Verification items for this drawing (mm, ordinates from the low corner). A direction names the side the tool comes from. Coordinates: 2 decimals unless noted, no trailing zeros. Write each loop counter-clockwise with the first axis right and the second up, starting at its lowest first coordinate (ties: lowest second). Pieces come first, ordered by that corner, then holes. Notation, with made-up numbers: M -14,59 L 34,59 A19 ccw 34,93 Z; hole C -0.75,67.5 d7. An arc over 180 degrees is marked long. Write each question's results on one line, items separated by ' | '.
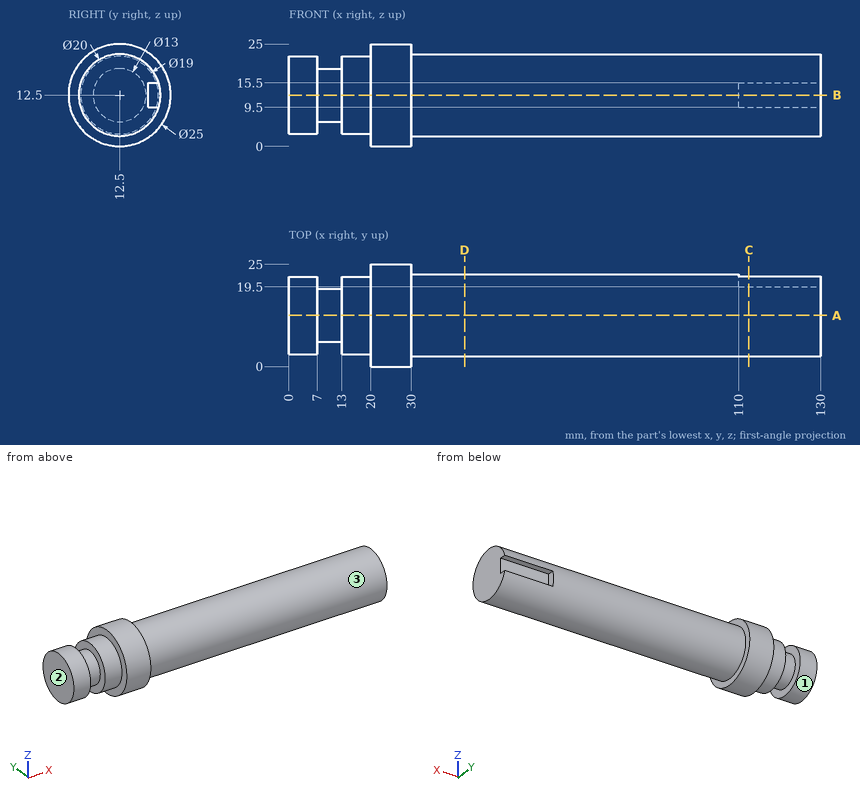
Q1. Sectioned sample at B-B on z = 12.5. Record the cut outline in (x, y).
Geometry check:
outline: M 0,3 L 7,3 L 7,6 L 13,6 L 13,3 L 20,3 L 20,0 L 30,0 L 30,2.5 L 130,2.5 L 130,19.5 L 110,19.5 L 110,22.5 L 30,22.5 L 30,25 L 20,25 L 20,22 L 13,22 L 13,19 L 7,19 L 7,22 L 0,22 Z
Q2. Sectioned sample at C-C on x = 112.5. Record the cut outline in (y, z), and give its area (3 significant figures).
Geometry check:
outline: M 19.5,9.5 L 19.5,15.5 L 22.04,15.5 A10 ccw long 22.04,9.5 Z | area: 297 mm2
Q3. Access from +Z, -Z, +X, -X, +Y, -Y to the whole of each face (thin tool, end or side, straight path). Record for the marked faces 1, 2 and 3.
Geometry check:
face 1: -X | face 2: +Z, -Z, -X, +Y, -Y | face 3: +X
Q4. Sectioned sample at A-A on y = 12.5. Record the cut outline in (x, z).
Geometry check:
outline: M 0,3 L 7,3 L 7,6 L 13,6 L 13,3 L 20,3 L 20,0 L 30,0 L 30,2.5 L 130,2.5 L 130,22.5 L 30,22.5 L 30,25 L 20,25 L 20,22 L 13,22 L 13,19 L 7,19 L 7,22 L 0,22 Z
Q5. Sectioned sample at D-D on x = 43. Record the cut outline in (y, z).
Geometry check:
outline: C 12.5,12.5 d20
Q6. Scan lines: probe 1 along X at (y, z) = (8, 7.75); probe 2 along Y at (x, z) = (24, 12.75); probe 3 along X at (y, z) = (19.25, 4). Record each from-to range of solid material in increasing order.
Geometry check:
probe 1: x = 0 to 7, 13 to 130 | probe 2: y = 0 to 25 | probe 3: x = 20 to 30
Q7. Depth check by flat-ended pin: P1, Ø4, axis at x = 55, y = 9, coming from the -Z side; P2, Ø3.5, axis at y = 20.5, z = 13, coming from the +X side; P3, Ø0.8, axis at x = 117, y = 20.5, coming from the -Z side; P4, Ø4, axis at x = 26.5, y = 17, coming from the -Z side. Enter the tip coordinate at first touch or a pass-through.
Geometry check:
P1: stops at z = 2.61 | P2: stops at x = 130 | P3: stops at z = 6 | P4: stops at z = 0.25
